Can you work these out from the model? Positions are in its coordinate system, mm. Face numbers are marked on the shaded views. A direction names the side the tool comes from. Round coordinates to 2 decimals unless told otherwise and drop trailing zeros. Loops run counter-clockwise (first coordinate to the right, second up) from the corner with the lowest first, then second, coordinate; pieces in that order, holes last. Notation, with made-up numbers: (83.5, 12) -> (115.5, 12) arc R25 ccw to (115.5, 30) -> close; hole circle Ø2 at (85.25, -4.5). An arc over 180 degrees is marked (long way). Write item = value, one per line.
from build123d import *

# Parameters (mm, degrees)
AXIAL_HOLE_M5_CLEARANCE_D           = 5.5
AXIAL_HOLE_M5_CLEARANCE_DEPTH       = 36.347633298
AXIAL_HOLE_M5_CLEARANCE_CSINK_D     = 5.55
AXIAL_HOLE_M5_CLEARANCE_CSINK_ANGLE = 100
AXIAL_HOLE_M5_CLEARANCE_TIP         = 1.652366702


with BuildPart() as part:
    # Shaft Profile Sketch → Stepped Shaft Revolve (revolve)
    with BuildSketch(Plane.XY, mode=Mode.PRIVATE) as stepped_shaft_revolve_sk:
        Polygon((0, 0), (0, 10), (7, 10), (7, 8), (10, 8), (10, 13), (28, 13), (28, 10), (42, 10), (42, 8), (55, 8), (55, 6), (72, 6), (72, 4), (82, 4), (82, 0), align=None)
    revolve(stepped_shaft_revolve_sk.sketch.rotate(Axis((-602.792603174, 0, 0), (1, 0, 0)), 90), axis=Axis((-602.792603174, 0, 0), (1, 0, 0)))

    # Axial Hole M5 Clearance
    with Locations(Plane(origin=(0, 0, 0), x_dir=(0, 0, -1), z_dir=(-1, 0, 0))):
        with Locations((0, 0)):
            CounterSinkHole(AXIAL_HOLE_M5_CLEARANCE_D / 2, AXIAL_HOLE_M5_CLEARANCE_CSINK_D / 2, depth=AXIAL_HOLE_M5_CLEARANCE_DEPTH, counter_sink_angle=AXIAL_HOLE_M5_CLEARANCE_CSINK_ANGLE)
            with Locations((0, 0, -(AXIAL_HOLE_M5_CLEARANCE_DEPTH + AXIAL_HOLE_M5_CLEARANCE_TIP / 2))):  # 118° drill point
                Cone(0, AXIAL_HOLE_M5_CLEARANCE_D / 2, AXIAL_HOLE_M5_CLEARANCE_TIP, mode=Mode.SUBTRACT)


solid = part.part
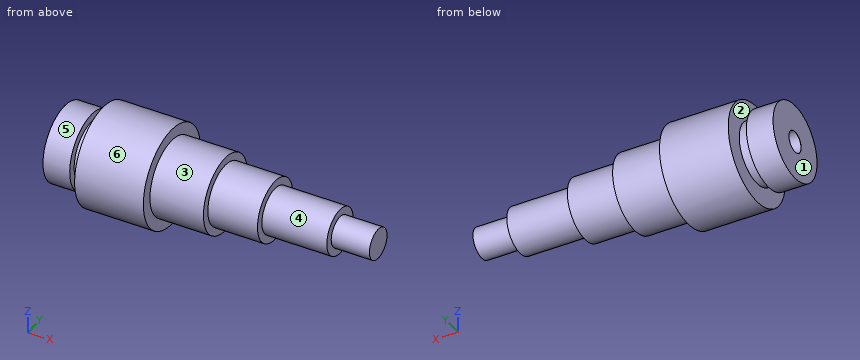
1. Suppose I cut it at A-A, the plane x = 22. List the corners of the cut face in (y, z) for me, and give its area (3 significant figures).
Entries:
outline = circle Ø26 at (0, 0); hole circle Ø5.5 at (0, 0)
area = 507 mm²
2. We'd pull the mould along X, two halves only. Please class the marked faces 1, 2 and 3: released by +X, released by -X, zero draft, split by the parting line, or undercut.
Entries:
face_1 = released by -X
face_2 = undercut
face_3 = zero draft
3. I need wall thicknesses on line 1 (X direction, y = -5, z = -6.5); line 2 (Y direction, x = 11, z = 0); line 3 (Y direction, x = 29, z = 0). Which ranges of each line are inside material? Lowest first, please. Write a range as [from, to].
Entries:
line_1 = [0, 7], [10, 42]
line_2 = [-13, -2.75], [2.75, 13]
line_3 = [-10, -2.75], [2.75, 10]
4. I'm going to push flat-ended pins straight in: pin 1 (8 mm diameter, centred on x = 51, z = -9, fed in from +Y) (3 decimals); pin 2 (8 mm diameter, centred on x = 43.5, y = -10, fed in from -Z); pin 3 (5 mm diameter, centred on x = 54, z = 1, fed in from -Y). Where does each tip first touch, or does it pass through?
Entries:
pin_1 = 6.245
pin_2 = -7.77
pin_3 = -8
5. For the marked faces 4, 5 and 6, which set-ups out of +Z, -Z, +X, -X, +Y, -Y let a thin tool reach every point of the face, with its end or its side?
Entries:
face_4 = +X
face_5 = -X
face_6 = +X, -X
6. Suppose I cut it at B-B, the plane y = -10.75. List the corners of the cut face in (x, z) for me, and give its area (3 significant figures).
Entries:
outline = (10, -7.31) -> (28, -7.31) -> (28, 7.31) -> (10, 7.31) -> close
area = 263 mm²
